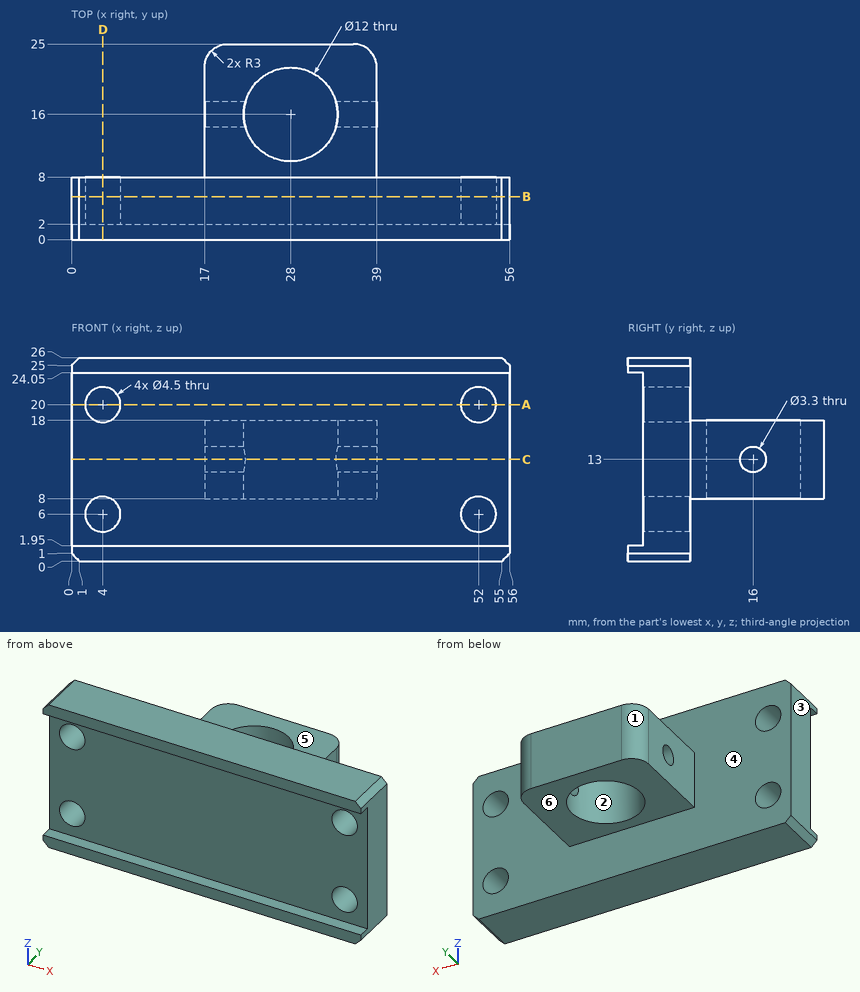
Geometry check sheet. Reference: drawing and pictorial views, mm from the part's lowest x, y, z. A direction names the side the tool comes from. Round coordinates to 2 decimals unless told otherwise and drop trailing zeros. Write each loop counter-clockwise with the first axis right and the second up, starting at its lowest first coordinate (ties: lowest second). Pieces come first, ordered by that corner, then holes. Notation, with made-up numbers: (-34, 71.5) -> (1, 71.5) arc R10 cw to (1, 84.5) -> close; hole circle Ø7 at (38.25, 69). An arc over 180 degrees is marked (long way). Put each result on its own line as item: value.
1) Cross-section at B-B, the plane y = 5.5. Enter the section's corners in (x, z).
Recorded:
outline: (0, 1) -> (1, 0) -> (55, 0) -> (56, 1) -> (56, 25) -> (55, 26) -> (1, 26) -> (0, 25) -> close; hole circle Ø4.5 at (4, 6); hole circle Ø4.5 at (4, 20); hole circle Ø4.5 at (52, 6); hole circle Ø4.5 at (52, 20)
2) Release check for a two-part mould opening along Y. For the marked faces 1, 2 and 3 record: pulls with the +Y half, pulls with the -Y half, needs draft (parallel to the pull), parting line crosses it, or undercut.
Recorded:
face 1: pulls with the +Y half
face 2: undercut
face 3: needs draft
3) Thickness scan on probe 1 along Z at (x, y) = (4, 4.4); probe 2 along Y at (x, z) = (19.95, 13); probe 3 along Y at (x, z) = (53, 22.5). Record the ranges inside material, lowest first. Write a range as from..to.
Recorded:
probe 1: z = 0..3.75, 8.25..17.75, 22.25..26
probe 2: y = 2..14.35, 17.65..25
probe 3: y = 2..8
4) Cross-section at A-A, the plane z = 20. Enter the section's corners in (x, y).
Recorded:
outline: (0, 2) -> (1.75, 2) -> (1.75, 8) -> (0, 8) -> close; (6.25, 2) -> (49.75, 2) -> (49.75, 8) -> (6.25, 8) -> close; (54.25, 2) -> (56, 2) -> (56, 8) -> (54.25, 8) -> close
5) Cross-section at D-D, the plane x = 4. Enter the section's corners in (y, z).
Recorded:
outline: (0, 0) -> (8, 0) -> (8, 3.75) -> (2, 3.75) -> (2, 1.95) -> (0, 1.95) -> close; (0, 24.05) -> (2, 24.05) -> (2, 22.25) -> (8, 22.25) -> (8, 26) -> (0, 26) -> close; (2, 8.25) -> (8, 8.25) -> (8, 17.75) -> (2, 17.75) -> close
6) Access from +Z, -Z, +X, -X, +Y, -Y to the whole of each face (thin tool, end or side, straight path). Record for the marked faces 4, 5 and 6.
Recorded:
face 4: +Y
face 5: +Z, +X, -X, +Y
face 6: -Z, +X, -X, +Y
7) Depth check by flat-ended pin: P1, Ø8.5, axis at x = 28.5, y = 17.5, coming from the -Z side; P2, Ø10, axis at x = 41.5, y = 20.5, coming from the +Z side; P3, Ø1.5, axis at y = 9.5, z = 16.5, coming from the -X side; P4, Ø12, axis at x = 37, y = 18.5, coming from the -Z side. Enter the tip coordinate at first touch or a pass-through.
Recorded:
P1: passes through
P2: stops at z = 18
P3: stops at x = 17
P4: stops at z = 8
8) Cross-section at C-C, the plane z = 13. Enter the section's corners in (x, y), plus the area to 3 significant figures.
Recorded:
outline: (0, 2) -> (56, 2) -> (56, 8) -> (39, 8) -> (39, 14.35) -> (33.77, 14.35) arc R6 cw to (22.23, 14.35) -> (17, 14.35) -> (17, 8) -> (0, 8) -> close; (17, 17.65) -> (22.23, 17.65) arc R6 cw to (33.77, 17.65) -> (39, 17.65) -> (39, 22) arc R3 ccw to (36, 25) -> (20, 25) arc R3 ccw to (17, 22) -> close
area: 560 mm2
